Work out the finished part from the listing and answer in its coordinate system (mm). A direction names the side the tool comes from. Round coordinates to 2 decimals unless told otherwise and drop trailing zeros. Loops run counter-clockwise (first coordinate to the right, second up) from the corner with the lowest first, then second, coordinate; pieces in that order, holes last. Notation, with made-up numbers: (79, 22.5) - (126, 22.5) arc R34 ccw to (126, 54.5) - close; hole circle Ø8 at (84, 65.25). An arc over 180 degrees is marked (long way). Answer as CSV lines item,"result". Start each with the question number.
Q1. The mould has two halves that part along X. Classify faces 1 (the face through (12, 10, -40)), 2 (the face through (0, 4, -15)), 3 (the face through (24, 10, -39)), 4 (the face through (11, 10, -32)): +X half, -X half, draft (parallel to the pull), parting line (faces both ways), or undercut.
Q2. Each of these flat-tipped pins is pushed along its axis until it touches: pin 1 Ø3 at (x, y) = (6.5, -5.5) entering from -Z; pin 2 Ø12.5 at (x, z) = (16.5, -23) entering from -Y. Where does it stop, or does it pass through?
Q3. Section D-D on z = -9 is taken. Write down the section's boundary in (x, y).
Q4. For faces 5 (the face through (13, -13, -15)), 6 (the face through (2.381, -15.008, -7.395)), determine the directions among +Z, -Z, +X, -X, +Y, -Y from which every point of the face is accessible in a straight line to the end or side of a thin tool.
Q5. Section A-A on z = -30 is taken. Write down the section's boundary in (x, y), then the cut area to 3 significant figures.
Q6. Section C-C on x = 5 is taken. Write down the section's boundary in (y, z), then the cut area to 3 significant figures.
Q7. Section B-B on y = 14 is taken. Write down the section's boundary in (x, z), then the cut area to 3 significant figures.
Q8. Straight lines are drawn through the part: L1, parallel to Y at x = 20, z = -6.5; L2, parallel to Z at x = 12.5, y = 14; L3, parallel to X at y = 12, z = -30. For each, find the intervals that lie inside material, in ascending order. Write a range as [from, to].
```python
from build123d import *

# Parameters (mm, degrees)
SKETCH_1_W           = 25
SKETCH_1_H           = 40
EXTRUDE_1_DEPTH      = 20
CHAMFER_1_SIZE       = 2
HOLE_WIZARD_M6_1_D   = 5
SKETCH_6_W           = 15
SKETCH_6_H           = 25
EXTRUDE_2_DEPTH      = 25
HOLE_WIZARD_M6_1_2_D = 6.6
CHAMFER_2_SIZE       = 2


with BuildPart() as part:
    # 草图1 → 凸台-拉伸1 (new body)
    with BuildSketch(Plane(origin=(0, 0, 0), x_dir=(1, 0, 0), z_dir=(0, 1, 0))):
        with Locations((12.5, 20)):
            Rectangle(SKETCH_1_W, SKETCH_1_H)
    extrude(amount=EXTRUDE_1_DEPTH)

    # 倒角1
    chamfer_1_edges = [part.edges().sort_by_distance(p)[0] for p in [
        (0, 10, -40),
        (25, 10, -40),
    ]]
    chamfer(chamfer_1_edges, length=CHAMFER_1_SIZE)

    # Hole Wizard M6 _1 (through all)
    with Locations(Plane(origin=(0, 0, 0), x_dir=(-1, 0, 0), z_dir=(0, -1, 0))):
        with Locations((-12.5, 30)):
            Hole(HOLE_WIZARD_M6_1_D / 2)

    # 草图6 → 凸台-拉伸2 (add)
    with BuildSketch(Plane(origin=(25, 0, 0), x_dir=(0, 0, -1), z_dir=(1, 0, 0))):
        with Locations((7.5, -12.5)):
            Rectangle(SKETCH_6_W, SKETCH_6_H)
    extrude(amount=-EXTRUDE_2_DEPTH)

    # Hole Wizard M6 _1 2 (through all)
    with Locations(Plane(origin=(0, 0, -15), x_dir=(-1, 0, 0), z_dir=(0, 0, -1))):
        with Locations((-20, -13), (-5, -13)):
            Hole(HOLE_WIZARD_M6_1_2_D / 2)

    # 倒角2
    chamfer_2_edges = [part.edges().sort_by_distance(p)[0] for p in [
        (25, -25, -7.5),
        (0, -25, -7.5),
    ]]
    chamfer(chamfer_2_edges, length=CHAMFER_2_SIZE)


solid = part.part
```
Findings:
1,face 1,"draft"
1,face 2,"-X half"
1,face 3,"+X half"
1,face 4,"undercut"
2,pin 1,"stops at z = -15"
2,pin 2,"stops at y = 0"
3,outline,"(0, -23) - (2, -25) - (23, -25) - (25, -23) - (25, 20) - (0, 20) - close; hole circle Ø6.6 at (5, -13); hole circle Ø6.6 at (20, -13)"
4,face 5,"-Z, +X, -X, -Y"
4,face 6,"+Z, -Z"
5,outline,"(0, 0) - (10, 0) - (10, 20) - (0, 20) - close; (15, 0) - (25, 0) - (25, 20) - (15, 20) - close"
5,area,"400 mm^2"
6,outline,"(-25, -15) - (-16.3, -15) - (-16.3, 0) - (-25, 0) - close; (-9.7, -15) - (0, -15) - (0, -40) - (20, -40) - (20, 0) - (-9.7, 0) - close"
6,area,"1,080 mm^2"
7,outline,"(0, -38) - (2, -40) - (23, -40) - (25, -38) - (25, 0) - (0, 0) - close; hole circle Ø5 at (12.5, -30)"
7,area,"976 mm^2"
8,L1,"y = [-25, -16.3], [-9.7, 20]"
8,L2,"z = [-40, -32.5], [-27.5, 0]"
8,L3,"x = [0, 10], [15, 25]"
